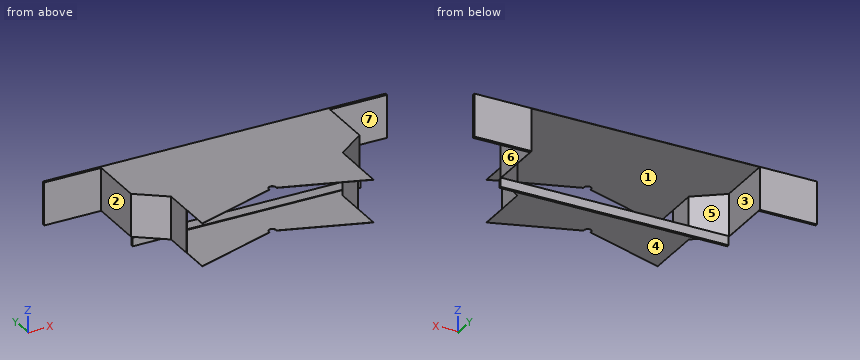
```python
from build123d import *

# Parameters (mm, degrees)
EXTRUDE_1_DEPTH     = 0.6
EXTRUDE_2_DEPTH     = 150
EXTRUDE_START       = -0.6
EXTRUDE_3_DEPTH     = 0.6
EXTRUDE_4_DEPTH     = 0.6
CUT_EXTRUDE_1_DEPTH = 569.863461773
EXTRUDE_5_DEPTH     = 100
SKETCH_9_W          = 150
SKETCH_9_H          = 7.683379221
EXTRUDE_6_DEPTH     = 200
SKETCH_11_W         = 150
SKETCH_11_H         = 9.400930001
EXTRUDE_7_DEPTH     = 200
EXTRUDE_10_DEPTH    = 2
SKETCH_16_W         = 799.99994366
SKETCH_16_H         = 30
EXTRUDE_12_DEPTH    = 8


with BuildPart() as part:
    # 草图1 → 凸台-拉伸1 (new body)
    with BuildSketch(Plane.XY):
        with BuildLine():
            Line((300, 0), (300, 230))
            Line((300, 230), (-300, 230))
            Line((-300, 230), (-300, 0))
            Line((-300, 0), (-9.486832981, 96.83772234))
            ThreePointArc((-9.486832981, 96.83772234), (0, 110), (9.486832981, 96.83772234))
            Line((9.486832981, 96.83772234), (300, 0))
        make_face()
    extrude(amount=EXTRUDE_1_DEPTH)

    # 草图4 → 凸台-拉伸2 (add)
    with BuildSketch(Plane(origin=(0, 0, 0), x_dir=(-1, 0, 0), z_dir=(0, 0, -1))):
        Polygon((-400, 375), (-400, 275), (-300, 200.300723127), (-300, 200), (-300, 100), (-300.6, 100), (-300.6, 200), (-400.600347155, 274.699536196), (-400.600347155, 375), align=None)
        Polygon((300, 100), (300.6, 100), (300.6, 200), (400.600347155, 274.699536196), (400.600347155, 375), (400, 375), (400, 275), (300, 200.300723127), (300, 200), align=None)
    extrude(amount=-EXTRUDE_2_DEPTH)

    # 草图5 → 凸台-拉伸3 (add)
    with BuildSketch(Plane.XY.offset(150).offset(EXTRUDE_START)):
        with BuildLine():
            Line((-300, 0), (-300, 100))
            Line((-300, 100), (-300.6, 100))
            Line((-300.6, 100), (-300.6, 200))
            Line((-300.6, 200), (-400.600347155, 274.699536196))
            Line((-400.600347155, 274.699536196), (-400.600347155, 375))
            Line((-400.600347155, 375), (400.600347155, 375))
            Line((400.600347155, 375), (400.600347155, 274.699536196))
            Line((400.600347155, 274.699536196), (300.6, 200))
            Line((300.6, 200), (300.6, 115))
            Line((300.6, 115), (300, 115))
            Line((300, 115), (300, 0))
            Line((300, 0), (9.486832981, 96.83772234))
            ThreePointArc((9.486832981, 96.83772234), (0, 110), (-9.486832981, 96.83772234))
            Line((-9.486832981, 96.83772234), (-300, 0))
        make_face()
    extrude(amount=EXTRUDE_3_DEPTH)

    # 草图6 → 凸台-拉伸4 (add)
    with BuildSketch(Plane(origin=(0, 0, 0), x_dir=(-1, 0, 0), z_dir=(0, 0, -1))):
        with BuildLine():
            Line((-300, 230), (-340.599999933, 230))
            Line((-340.599999933, 230), (-300.6, 200))
            ThreePointArc((-300.6, 200), (-300.207294902, 199.964589803), (-300, 200.3))
            Line((-300, 200.3), (-300, 230))
        make_face()
        Polygon((300, 230), (343.651844708, 232.159416678), (300.6, 200), (300, 200.300723127), align=None)
    extrude(amount=-EXTRUDE_4_DEPTH)

    # 草图7 → 切除-拉伸1 (cut, through all)
    with BuildSketch(Plane.XY.offset(150)):
        with BuildLine():
            Line((-12.5, 100), (-12.5, 86.103683602))
            Line((-12.5, 86.103683602), (12.5, 86.103683602))
            Line((12.5, 86.103683602), (12.5, 100))
            ThreePointArc((12.5, 100), (0, 112.5), (-12.5, 100))
        make_face()
    extrude(amount=-CUT_EXTRUDE_1_DEPTH, mode=Mode.SUBTRACT)

    # 草图8 → 凸台-拉伸5 (add)
    with BuildSketch(Plane(origin=(0, 375, 0), x_dir=(1, 0, 0), z_dir=(0, 1, 0))):
        Polygon((-400.600347155, 0), (-400, 0), (-400, -149.4), (400, -149.4), (400, 0), (400.600347155, 0), (400.600347155, -149.4), (400.600347155, -150), (-400, -150), (-400.600347155, -150), align=None)
    extrude(amount=EXTRUDE_5_DEPTH)

    # 草图9 → 凸台-拉伸6 (add)
    with BuildSketch(Plane.ZY.offset(400.600347155)):
        with Locations((75, 471.15831039)):
            Rectangle(SKETCH_9_W, SKETCH_9_H)
    extrude(amount=EXTRUDE_6_DEPTH)

    # 草图11 → 凸台-拉伸7 (add)
    with BuildSketch(Plane(origin=(400.600347155, 0, 0), x_dir=(0, 0, -1), z_dir=(1, 0, 0))):
        with Locations((-75, 470.299535)):
            Rectangle(SKETCH_11_W, SKETCH_11_H)
    extrude(amount=EXTRUDE_7_DEPTH)

    # 草图12 → 凸台-拉伸10 (add)
    with BuildSketch(Plane(origin=(0, 0, 0), x_dir=(-1, 0, 0), z_dir=(0, 0, -1))):
        Polygon((-339.758452982, 230), (-400, 275), (400.600347155, 274.699536196), (342.578162478, 232.106302604), align=None)
    extrude(amount=-EXTRUDE_10_DEPTH)

    # 草图16 → 凸台-拉伸12 (add)
    with BuildSketch(Plane(origin=(-0.103150629, 274.84984204, 0), x_dir=(0.9999999295756685, 0.00037529809229504854, 0), z_dir=(-0.0003752980922950485, 0.9999999295756684, 0))):
        with Locations((0.178266594, 15)):
            Rectangle(SKETCH_16_W, SKETCH_16_H)
    extrude(amount=-EXTRUDE_12_DEPTH)


solid = part.part
```
The model under review builds one solid part; all positions refer to its coordinate system, in mm. Face numbers are marked on the shaded views. A direction names the side the tool comes from. Round coordinates to 2 decimals unless told otherwise and drop trailing zeros. Write each loop counter-clockwise with the first axis right and the second up, starting at its lowest first coordinate (ties: lowest second). Pieces come first, ordered by that corner, then holes.
(1) We need section D-D on x = -366. Give the boundary of the cut face in (y, z).
(2) Wall thickness on L1, parallel to X at y = 407.5, z = 116.5; L2, parallel to X at y = 132, z = 61; L3, parallel to Z at x = 136.5, y = 249: over which ranges is each line inside the solid? List them lowest first.
(3) Insertion check: pin 1 (12 mm diameter, centred on y = 207, z = 104.5, fed in from +X); pin 2 (2 mm diameter, centred on y = 132.5, z = 44.5, fed in from -X); pin 3 (0.5 mm diameter, centred on y = 98.5, z = 0, fed in from +X). Each pin has a flat end and moves straight along its axis. Give the tip position at first contact, or say it passes through.
(4) We need section A-A on z = 123.5. Give the boundary of the cut face in (x, y), and give its area (3 significant figures).
(5) We need section C-C on y = 214.5. Give the boundary of the cut face in (x, z).
(6) We need section B-B on x = -197. Give the boundary of the cut face in (y, z), and give its area (3 significant figures).
(7) Mouldability with a two-part tool opening along X and no side actions: class the marked faces 5, 6 and 7 as +X half, -X half, draft (parallel to the pull), parting line (faces both ways), or undercut.
(8) Machinability: for the marked faces 1, 2, 3 and 4, which of the approach directions +Z, -Z, +X, -X, +Y, -Y give a long, thin tool a straight path to every point of the face, cutting with its end or side? Answer none if there is none.
Findings below:
1. outline: (248.85, 0) - (266.71, 0) - (266.71, -30) - (274.71, -30) - (274.71, 2) - (249.6, 2) - (249.6, 149.4) - (475, 149.4) - (475, 150) - (248.85, 150) - close
2. L1: x = -400.6 to -400, 400 to 400.6
2. L2: x = -300.6 to -300, 300 to 300.6
2. L3: z = 0 to 2, 149.4 to 150
3. pin 1: stops at x = 318
3. pin 2: stops at x = -300.6
3. pin 3: stops at x = 300
4. outline: (-600.6, 467.32) - (-400.6, 467.32) - (-400.6, 274.7) - (-300.6, 200) - (-300.6, 100) - (-300, 100) - (-300, 200.3) - (-400, 275) - (-400, 475) - (-600.6, 475) - close; (300, 100) - (300.6, 100) - (300.6, 200) - (400.6, 274.7) - (400.6, 465.6) - (600.6, 465.6) - (600.6, 475) - (400, 475) - (400, 275) - (300, 200.3) - close
4. area: 3,930 mm2
5. outline: (-320.01, 0) - (320.01, 0) - (320.01, 150) - (-320.01, 150) - close; hole (-319.01, 0.6) - (319.01, 0.6) - (319.01, 149.4) - (-319.01, 149.4) - close
6. outline: (34.33, 0) - (230, 0) - (230, 0.6) - (34.33, 0.6) - close; (34.33, 149.4) - (475, 149.4) - (475, 150) - (34.33, 150) - close; (231.66, 0) - (266.78, 0) - (266.78, -30) - (274.78, -30) - (274.78, 2) - (231.66, 2) - close
6. area: 708 mm2
7. face 5: undercut
7. face 6: +X half
7. face 7: draft
8. face 1: +Y
8. face 2: +Z, -Z, -X, -Y
8. face 3: -Z, +Y
8. face 4: -Z, +X, -X, -Y
